Design review of the part built by this model. Coordinates are the model's own, in mm. A direction names the side the tool comes from. Give positions to 0.01 mm unless a question says otherwise; leave off trailing zeros. Loops run counter-clockwise (first coordinate to the right, second up) from the corner with the lowest first, then second, coordinate; pieces in that order, holes last. Notation, with made-up numbers: M -32,37 L 9,37 A29 cw 9,58 Z; hole C -4.75,4.5 d2. An arc over 180 degrees is marked long. Use one line per item in the form item = value. Start each with the question number.
from build123d import *

# Parameters (mm, degrees)
EXTRUDE_1_DEPTH = 100
REVOLVE_1_ANGLE = 90


with BuildPart() as part:
    # 草图1 → 凸台-拉伸1 (new body)
    with BuildSketch(Plane.XY):
        with BuildLine():
            Line((0, 0), (0, -80))
            Line((0, -80), (-20, -80))
            ThreePointArc((-20, -80), (-60, -40), (-20, 0))
            Line((-20, 0), (0, 0))
        make_face()
    extrude(amount=-EXTRUDE_1_DEPTH)

    # 草图2 → 旋转1 (revolve)
    with BuildSketch(Plane(origin=(0, 0, 0), x_dir=(0, 0, -1), z_dir=(1, 0, 0))):
        with BuildLine():
            Line((100, 20), (100, -100))
            ThreePointArc((100, -100), (160, -40), (100, 20))
        make_face()
    revolve(axis=Axis((0, 20, -100), (0, 1, 0)), revolution_arc=REVOLVE_1_ANGLE)


solid = part.part
Q1. Take a section at A-A on x = -14. Give the boundary of the cut face in (y, z), plus the area to 3 significant figures.
Q2. Clearance check with flat-ended pins moving along their axes: pin 1 Ø1 at (x, z) = (-32.5, -132.5) entering from +Y; pin 2 Ø12 at (y, z) = (-47, -60) entering from -X; pin 3 Ø1.5 at (x, z) = (-28.5, -80) entering from -Y. State where each tip first meets the part, or that it passes through.
Q3. Take a section at C-C on y = -77. Give the boundary of the cut face in (x, z).
Q4. Take a section at D-D on x = -30. Give the boundary of the cut face in (y, z).
Q5. Wall thickness on probe 1 along Y at (x, z) = (-3.5, -87.5); probe 2 along X at (y, z) = (-40.5, -11); probe 3 along Y at (x, z) = (-29, -80.5): over which ranges is each line inside the solid? List them lowest first.
Q6. For faces 1 (the flat face through (-10, 0, -49)), 2 (the flat face through (-10, -80, -49)), 3 (the flat face through (-23, 3, -100)), list the 3-axis set-ups (+Z, -Z, +X, -X, +Y, -Y) from which the entire face can be reached by the end or side of a thin tool; tool diameter is ignored.
Q7. Take a section at B-B on z = -79. Give the boundary of the cut face in (x, y).
Response values:
q1.outline = M -98.34,-100 A58.34 ccw 18.34,-100 L 0,-100 L 0,0 L -80,0 L -80,-100 Z
q1.area = 13,300 mm^2
q2.pin_1 = -0.84
q2.pin_2 = -59.99
q2.pin_3 = -79.24
q3.outline = M -47.23,-100 A47.23 ccw 0,-147.23 L 0,0 L -35.2,0 L -35.2,-100 Z
q4.outline = M -91.96,-100 A51.96 ccw 11.96,-100 L -1.27,-100 L -1.27,0 L -78.73,0 L -78.73,-100 Z
q5.probe_1 = -80 to 0
q5.probe_2 = -60 to 0
q5.probe_3 = -78.97 to -1.03
q6.face_1 = +Z, +X, -X, +Y
q6.face_2 = +Z, +X, -X, -Y
q6.face_3 = +Z, -X, +Y
q7.outline = M -20,-80 L 0,-80 L 0,0 L -20,0 A40 ccw Z
